Verification items for this drawing (mm, ordinates from the low corner). A direction names the side the tool comes from. Round coordinates to 2 decimals unless told otherwise and drop trailing zeros. Write each loop counter-clockwise with the first axis right and the second up, starting at its lowest first coordinate (ties: lowest second). Pieces come first, ordered by that corner, then holes. Notation, with made-up numbers: M -35,62.25 L -29,62.25 A13 ccw -29,70.25 Z; hole C 66,-12 d1. An arc over 180 degrees is marked long. Write each question's results on one line, items separated by ' | '.
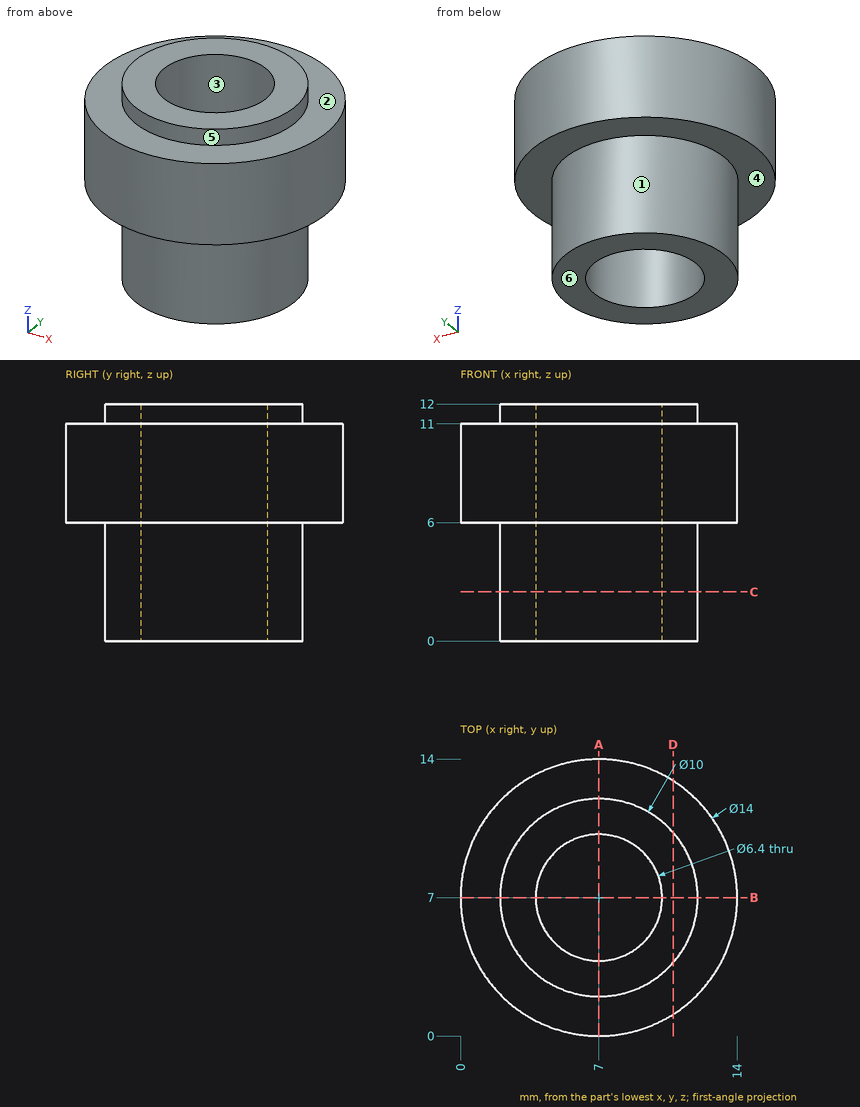
1) Depth check by flat-ended pin: P1, Ø1.5, axis at y = 6, z = 9.5, coming from the -X side; P2, Ø5, axis at x = 7, y = 7, coming from the -Z side; P3, Ø5, axis at y = 9.5, z = 4, coming from the -X side; P4, Ø4, axis at x = 8.5, z = 3.5, coming from the -Y side. Enter the tip coordinate at first touch or a pass-through.
Calculated:
P1: stops at x = 0 | P2: passes through | P3: stops at x = 0.07 | P4: stops at y = 2
2) Access from +Z, -Z, +X, -X, +Y, -Y to the whole of each face (thin tool, end or side, straight path). Record for the marked faces 4, 5 and 6.
Calculated:
face 4: -Z | face 5: +Z | face 6: -Z, +X, -X, +Y, -Y
3) Sectioned sample at C-C, the plane z = 2.5. Record the cut outline in (x, y), and give its area (3 significant figures).
Calculated:
outline: C 7,7 d10; hole C 7,7 d6.4 | area: 46.4 mm²
4) Sectioned sample at D-D, the plane x = 10.75. Record the cut outline in (y, z).
Calculated:
outline: M 1.09,6 L 3.69,6 L 3.69,0 L 10.31,0 L 10.31,6 L 12.91,6 L 12.91,11 L 10.31,11 L 10.31,12 L 3.69,12 L 3.69,11 L 1.09,11 Z
5) Sectioned sample at A-A, the plane x = 7. Record the cut outline in (y, z), and give its area (3 significant figures).
Calculated:
outline: M 0,6 L 2,6 L 2,0 L 3.8,0 L 3.8,12 L 2,12 L 2,11 L 0,11 Z; M 10.2,0 L 12,0 L 12,6 L 14,6 L 14,11 L 12,11 L 12,12 L 10.2,12 Z | area: 63.2 mm²
6) Draft check along X on the marked faces 1, 2 and 3. Enter one of: pulls with the +X half, pulls with the -X half, needs draft (parallel to the pull), parting line crosses it, or undercut.
Calculated:
face 1: parting line crosses it | face 2: needs draft | face 3: undercut
7) Material ranges on line 1 (Y direction, x = 7, z = 5); line 2 (Y direction, x = 7, z = 7); line 3 (X direction, y = 8.5, z = 9.5), recorded low to high. Write a range as [from, to].
Calculated:
line 1: y = [2, 3.8], [10.2, 12] | line 2: y = [0, 3.8], [10.2, 14] | line 3: x = [0.16, 4.17], [9.83, 13.84]
